```python
from build123d import *

# Parameters (mm, degrees)
SKETCH1_R           = 3
BOSS_EXTRUDE1_DEPTH = 20


with BuildPart() as part:
    # Sketch1 → Boss-Extrude1 (new body)
    with BuildSketch(Plane.XY):
        with BuildLine():
            Line((0, 7.5), (30, 7.5))
            ThreePointArc((30, 7.5), (37.5, 0), (30, -7.5))
            Line((30, -7.5), (0, -7.5))
            ThreePointArc((0, -7.5), (-7.5, 0), (0, 7.5))
        make_face()
        Circle(SKETCH1_R, mode=Mode.SUBTRACT)
        with Locations((30, 0)):
            Circle(SKETCH1_R, mode=Mode.SUBTRACT)
    extrude(amount=BOSS_EXTRUDE1_DEPTH)


solid = part.part
```
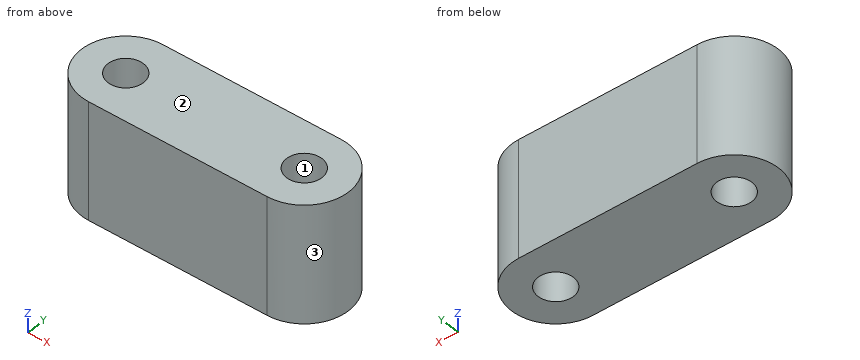
Here's how the part is built. I have some questions about the finished solid (model axes, mm). Face numbers are marked on the shaded views. Give positions to 0.01 mm unless a question says otherwise; leave off trailing zeros. Write each loop counter-clockwise with the first axis right and the second up, starting at its lowest first coordinate (ties: lowest second). Pieces come first, ordered by that corner, then holes. Notation, with made-up numbers: M -31,59.5 L -25,59.5 A6 cw -25,67.5 Z; hole C 1.5,-17 d8. An arc over 180 degrees is marked long. Put each result on its own line as item: value. Start each with the question number.
Item 1: Thinking about a two-plate mould opening in X: for the marked faces 1, 2 and 3, which applies, +X half, -X half, draft (parallel to the pull), parting line (faces both ways), or undercut?
Item 2: If we section it at C-C, the plane z = 5.75: Write out the boundary of the cut face in (x, y), then the cut area to 3 significant figures.
Item 3: If we section it at B-B, the plane x = -1.5: Write out the boundary of the cut face in (y, z), then the cut area to 3 significant figures.
Item 4: I need wall thicknesses on L1, parallel to Y at x = 0, z = 6.25; L2, parallel to X at y = -1, z = 6.75; L3, parallel to Y at x = 2, z = 15.25. Which ranges of each line are inside material? Lowest first, please. Write a range as from..to.
Item 5: If we section it at D-D, the plane x = 32.5: Write out the boundary of the cut face in (y, z), then the cut area to 3 significant figures.
Item 6: If we section it at A-A, the plane y = 0: Write out the boundary of the cut face in (x, z).
Item 7: Will these pins go through, and if not, where does the flat tip stop? pin 1 (2 mm diameter, centred on x = 25, y = 4.5, fed in from -Z); pin 2 (8 mm diameter, centred on y = -5.5, z = 16.5, fed in from -X); pin 3 (1.5 mm diameter, centred on y = -4.5, z = 12.5, fed in from -X); pin 4 (1 mm diameter, centred on y = -3, z = 8.5, fed in from +X).
Values:
1. face 1: undercut
1. face 2: draft
1. face 3: +X half
2. outline: M 0,-7.5 L 30,-7.5 A7.5 ccw 30,7.5 L 0,7.5 A7.5 ccw Z; hole C 0,0 d6; hole C 30,0 d6
2. area: 570 mm²
3. outline: M -7.35,0 L -2.6,0 L -2.6,20 L -7.35,20 Z; M 2.6,0 L 7.35,0 L 7.35,20 L 2.6,20 Z
3. area: 190 mm²
4. L1: -7.5..-3, 3..7.5
4. L2: -7.43..-2.83, 2.83..27.17, 32.83..37.43
4. L3: -7.5..-2.24, 2.24..7.5
5. outline: M -7.07,0 L -1.66,0 L -1.66,20 L -7.07,20 Z; M 1.66,0 L 7.07,0 L 7.07,20 L 1.66,20 Z
5. area: 217 mm²
6. outline: M -7.5,0 L -3,0 L -3,20 L -7.5,20 Z; M 3,0 L 27,0 L 27,20 L 3,20 Z; M 33,0 L 37.5,0 L 37.5,20 L 33,20 Z
7. pin 1: z = 0
7. pin 2: x = -7.35
7. pin 3: x = -6.5
7. pin 4: x = 37.07
